The listing builds one solid part. Answer for the finished solid, in the listing's coordinates (mm). Face numbers are marked on the shaded views. Coordinates: 2 decimals unless noted, no trailing zeros. Order: outer loops, then holes, each group sorted by start corner. A loop starts at its lowest first (then second) coordinate and runs counter-clockwise, first axis right, second up. Notation, with made-up numbers: (-6, -21) -> (25, -21) arc R27 ccw to (25, 6) -> close; hole circle Ø8 at (68.25, 12.25). An arc over 180 degrees is marked (long way). Answer in a Markdown table with one row per item.
```python
from build123d import *

# Parameters (mm, degrees)
SKETCH_1_W          = 160
SKETCH_1_H          = 60
EXTRUDE_1_DEPTH     = 10
HOLE_WIZARD_M20_1_D = 17.5
HOLE_WIZARD_M8_1_D  = 6.8


with BuildPart() as part:
    # 草图1 → 凸台-拉伸1 (new body)
    with BuildSketch(Plane.XY):
        Rectangle(SKETCH_1_W, SKETCH_1_H)
    extrude(amount=EXTRUDE_1_DEPTH)

    # M20 螺纹孔1 (through all)
    with Locations(Plane.XY.offset(10)):
        with Locations((-50, 0)):
            Hole(HOLE_WIZARD_M20_1_D / 2)

    # M8 螺纹孔1 (through all)
    with Locations(Plane.XY.offset(10)):
        with Locations((17.5, 21), (72.5, 21), (17.5, -21), (72.5, -21)):
            Hole(HOLE_WIZARD_M8_1_D / 2)


solid = part.part
```
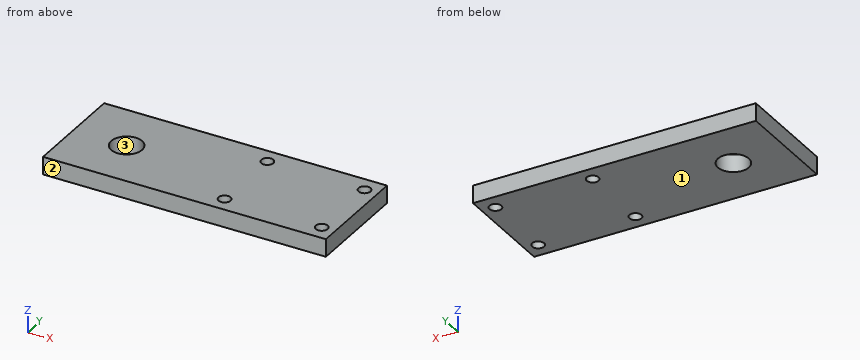
(1) Find the intervals of material crossed by line 1 along Y through (x, z) = (72.5, 5.5); line 2 along X through (y, z) = (-20, 7.75); line 3 along X through (y, z) = (-23, 6.5), in increasing order. Write a range as from..to.
Check values:
| item | result |
|---|---|
| line 1 | -30..-24.4, -17.6..17.6, 24.4..30 |
| line 2 | -80..14.25, 20.75..69.25, 75.75..80 |
| line 3 | -80..14.75, 20.25..69.75, 75.25..80 |
(2) A cutting plane is placed at C-C, the plane y = 21. Determine the outline of the cut face in (x, z), then the cut area to 3 significant figures.
Check values:
| item | result |
|---|---|
| outline | (-80, 0) -> (14.1, 0) -> (14.1, 10) -> (-80, 10) -> close; (20.9, 0) -> (69.1, 0) -> (69.1, 10) -> (20.9, 10) -> close; (75.9, 0) -> (80, 0) -> (80, 10) -> (75.9, 10) -> close |
| area | 1,460 mm² |
(3) Flat-ended cylindrical pins translate along their axes: pin 1 (4 mm diameter, centred on x = 72.5, y = 21, fed in from -Z); pin 2 (9 mm diameter, centred on x = 17.5, y = 21, fed in from +Z). Find the tip coordinate at first contact, or state that the pin passes through.
Check values:
| item | result |
|---|---|
| pin 1 | through |
| pin 2 | z = 10 |
(4) For a pull along Y with two mould halves and no side action, classify the marked faces 1, 2 and 3 as released by +Y, released by -Y, zero draft, split by the parting line, or undercut.
Check values:
| item | result |
|---|---|
| face 1 | zero draft |
| face 2 | released by -Y |
| face 3 | undercut |
(5) A cutting plane is placed at D-D, the plane x = 17.5. Determine the outline of the cut face in (y, z), then the cut area to 3 significant figures.
Check values:
| item | result |
|---|---|
| outline | (-30, 0) -> (-24.4, 0) -> (-24.4, 10) -> (-30, 10) -> close; (-17.6, 0) -> (17.6, 0) -> (17.6, 10) -> (-17.6, 10) -> close; (24.4, 0) -> (30, 0) -> (30, 10) -> (24.4, 10) -> close |
| area | 464 mm² |
(6) A cutting plane is placed at B-B, the plane x = -50. Determine the outline of the cut face in (y, z), then the cut area to 3 significant figures.
Check values:
| item | result |
|---|---|
| outline | (-30, 0) -> (-8.75, 0) -> (-8.75, 10) -> (-30, 10) -> close; (8.75, 0) -> (30, 0) -> (30, 10) -> (8.75, 10) -> close |
| area | 425 mm² |
(7) A cutting plane is placed at A-A, the plane y = 0. Determine the outline of the cut face in (x, z), then the cut area to 4 significant figures.
Check values:
| item | result |
|---|---|
| outline | (-80, 0) -> (-58.75, 0) -> (-58.75, 10) -> (-80, 10) -> close; (-41.25, 0) -> (80, 0) -> (80, 10) -> (-41.25, 10) -> close |
| area | 1,425 mm² |
